from build123d import *

# Parameters (mm, degrees)
SKETCH1_R           = 50
BOSS_EXTRUDE1_DEPTH = 5
FILLET1_R           = 5
SKETCH2_R           = 1.9
CUT_EXTRUDE1_DEPTH  = 5


with BuildPart() as part:
    # Sketch1 → Boss-Extrude1 (new body)
    with BuildSketch(Plane.XY):
        Circle(SKETCH1_R)
        with BuildLine():
            Line((30.504506916, 35.755769574), (0, 5.251262658))
            Line((0, 5.251262658), (-30.504506916, 35.755769574))
            ThreePointArc((-30.504506916, 35.755769574), (0, 47), (30.504506916, 35.755769574))
        make_face(mode=Mode.SUBTRACT)
        with BuildLine():
            Line((5.251262658, 0), (35.755769574, 30.504506916))
            ThreePointArc((35.755769574, 30.504506916), (47, 0), (35.755769574, -30.504506916))
            Line((35.755769574, -30.504506916), (5.251262658, 0))
        make_face(mode=Mode.SUBTRACT)
        with BuildLine():
            Line((0, -5.251262658), (30.504506916, -35.755769574))
            ThreePointArc((30.504506916, -35.755769574), (0, -47), (-30.504506916, -35.755769574))
            Line((-30.504506916, -35.755769574), (0, -5.251262658))
        make_face(mode=Mode.SUBTRACT)
        with BuildLine():
            Line((-5.251262658, 0), (-35.755769574, -30.504506916))
            ThreePointArc((-35.755769574, -30.504506916), (-47, 0), (-35.755769574, 30.504506916))
            Line((-35.755769574, 30.504506916), (-5.251262658, 0))
        make_face(mode=Mode.SUBTRACT)
    extrude(amount=BOSS_EXTRUDE1_DEPTH)

    # Fillet1
    fillet1_edges = [part.edges().sort_by_distance(p)[0] for p in [
        (-5.251262658, 0, 2.5),
        (-35.755769574, 30.504506916, 2.5),
        (-35.755769574, -30.504506916, 2.5),
        (35.755769574, -30.504506916, 2.5),
        (35.755769574, 30.504506916, 2.5),
        (5.251262658, 0, 2.5),
        (-30.504506916, -35.755769574, 2.5),
        (30.504506916, -35.755769574, 2.5),
        (0, -5.251262658, 2.5),
        (30.504506916, 35.755769574, 2.5),
        (-30.504506916, 35.755769574, 2.5),
        (0, 5.251262658, 2.5),
    ]]
    fillet(fillet1_edges, radius=FILLET1_R)

    # Sketch2 → Cut-Extrude1 (cut)
    with BuildSketch(Plane.XY.offset(5)):
        with Locations((5.656854249, -5.656854249)):
            Circle(SKETCH2_R)
        with Locations((5.656854249, 5.656854249)):
            Circle(SKETCH2_R)
        with Locations((-5.656854249, 5.656854249)):
            Circle(SKETCH2_R)
        with Locations((-5.656854249, -5.656854249)):
            Circle(SKETCH2_R)
    extrude(amount=-CUT_EXTRUDE1_DEPTH, mode=Mode.SUBTRACT)


solid = part.part
Verification items for the finished model (mm, model axes). Give positions to 0.01 mm unless a question says otherwise; leave off trailing zeros. Write each loop counter-clockwise with the first axis right and the second up, starting at its lowest first coordinate (ties: lowest second). Pieces come first, ordered by that corner, then holes. Notation, with made-up numbers: M 40,21 L 52,21 A19 ccw 52,35 Z; hole C 59.25,-35.5 d4. An arc over 180 degrees is marked long. Put each result on its own line as item: value. Start each with the question number.
1. Go/stop test with flat-tipped pins: pin 1 Ø5 at (x, y) = (5.66, -5.66) entering from -Z; pin 2 Ø2 at (y, z) = (12.5, 3) entering from +X; pin 3 Ø1.5 at (x, z) = (-5, 4) entering from -Y; pin 4 Ø2.5 at (x, y) = (5.66, 5.66) entering from +Z. Record where each tip stops, or that it passes through.
2. Section check A-A (x = 0). Record the cut outline in (y, z), and give its area (3 significant figures).
3. Section check C-C (z = 3.2). Give the number of separate pieces and of enclosed holes in the cut face, and give its area (3 significant figures).
4. Draft check along X on faces 1 (the face through (0, 0, 5)), 2 (the face through (-0.055, -7.323, 2.535)). Enter one of: +X half, -X half, draft (parallel to the pull), parting line (faces both ways), or undercut.
5. Section check D-D (y = 20). Record the cut outline in (x, z), and give its area (3 significant figures).
6. Scan lines: line 1 along Y through (x, z) = (-0.5, 0.35); line 2 along Y through (x, z) = (19, 4.3); line 3 along Y through (x, z) = (-27, 0.3). Record each from-to range of solid material in increasing order. Write a range as [from, to].
Answer list:
1. pin 1: z = 0
1. pin 2: x = 48.66
1. pin 3: y = -49.82
1. pin 4: through
2. outline: M -50,0 L -47,0 L -47,5 L -50,5 Z; M -7.32,0 L 7.32,0 L 7.32,5 L -7.32,5 Z; M 47,0 L 50,0 L 50,5 L 47,5 Z
2. area: 103 mm2
3. separate pieces: 1
3. enclosed holes: 8
3. area: 2,290 mm2
4. face 1: draft
4. face 2: undercut
5. outline: M -45.83,0 L -42.53,0 L -42.53,5 L -45.83,5 Z; M -25.25,0 L -14.75,0 L -14.75,5 L -25.25,5 Z; M 14.75,0 L 25.25,0 L 25.25,5 L 14.75,5 Z; M 42.53,0 L 45.83,0 L 45.83,5 L 42.53,5 Z
5. area: 138 mm2
6. line 1: [-50, -47], [-7.35, 7.35], [47, 50]
6. line 2: [-46.25, -42.99], [-24.25, -13.75], [13.75, 24.25], [42.99, 46.25]
6. line 3: [-42.08, -38.06], [-32.36, -21.75], [21.75, 32.36], [38.06, 42.08]
